from build123d import *

# Parameters (mm, degrees)
SKETCH_1_R      = 10
EXTRUDE_1_DEPTH = 12.5


with BuildPart() as part:
    # 草图1 → 凸台-拉伸1 (new, symmetric)
    with BuildSketch(Plane(origin=(0, 0, 0), x_dir=(1, 0, 0), z_dir=(0, 1, 0))):
        Polygon((0, 22.5), (-19.485571585, 11.25), (-19.485571585, -11.25), (0, -22.5), (19.485571585, -11.25), (19.485571585, 11.25), align=None)
        with Locations(Location((0, 0, 0), (0, 0, 270))):
            Circle(SKETCH_1_R, mode=Mode.SUBTRACT)
    extrude(amount=EXTRUDE_1_DEPTH, both=True)

    # 草图2 → 切除-旋转1 (revolve, cut)
    with BuildSketch(Plane(origin=(0, 0, 0), x_dir=(0, 0, -1), z_dir=(1, 0, 0))):
        with BuildLine():
            Line((-22.5, 10.5), (-22.5, 12.5))
            Line((-22.5, 12.5), (-17.5, 12.5))
            ThreePointArc((-17.5, 12.5), (-20.005385321, 11.513463302), (-22.5, 10.5))
        make_face()
    cut_revolve_1 = revolve(axis=Axis((0, 32.499694269, 0), (0, -1, 0)), mode=Mode.SUBTRACT)

    # 镜向1: 切除-旋转1 across plane
    add(cut_revolve_1.mirror(Plane.ZX), mode=Mode.SUBTRACT)


solid = part.part
Input: part model. Units: mm. Frame: model coordinates. Give positions to 0.01 mm unless a question says otherwise; leave off trailing zeros. Write each loop counter-clockwise with the first axis right and the second up, starting at its lowest first coordinate (ties: lowest second). Pieces come first, ordered by that corner, then holes. Notation, with made-up numbers: M 48,36.5 L 103,36.5 A7 cw 103,45.5 Z; hole C 88,-26.75 d9. An arc over 180 degrees is marked long. Use one line per item in the form item = value.
1. Mould query, pull axis X, two halves, no side actions, for faces 1 (the face through (8, 12.5, 8)), 2 (the face through (-19.486, 0, 0)), 3 (the face through (9.879, 0.164, -16.796)), 4 (the face through (-9.76, -0.18, -2.17)). Classes: released by +X, released by -X, zero draft, split by the parting line, or undercut.
Outcome:
face_1 = zero draft
face_2 = released by -X
face_3 = released by +X
face_4 = undercut
2. Cut plane A-A on y = 4. Return loops of the section in (x, z).
Outcome:
outline = M -19.49,-11.25 L 0,-22.5 L 19.49,-11.25 L 19.49,11.25 L 0,22.5 L -19.49,11.25 Z; hole C 0,0 d20
3. Ray query, L1, parallel to X at y = -3.5, z = 0; L2, parallel to Z at x = -5.5, y = -8.75; L3, parallel to X at y = 4, z = -3. Return the intervals inside material, ascending.
Outcome:
L1 = -19.49 to -10, 10 to 19.49
L2 = -19.32 to -8.35, 8.35 to 19.32
L3 = -19.49 to -9.54, 9.54 to 19.49
4. First-contact query: P1, Ø12, axis at x = -5.5, y = 1.5, coming from the +Z side; P2, Ø5, axis at x = -9.5, y = 6.5, coming from the +Z side. Flat tips, straight axial feed; report the tip coordinate or a pass-through.
Outcome:
P1 = 22.5
P2 = 18.46
